from build123d import *

# Parameters (mm, degrees)
SKETCH_1_W          = 150
SKETCH_1_H          = 110
EXTRUDE_1_DEPTH     = 2.5
SKETCH_2_R          = 33.915864145
CUT_EXTRUDE_1_DEPTH = 10


with BuildPart() as part:
    # 草图1 → 凸台-拉伸1 (new, symmetric)
    with BuildSketch(Plane.XY):
        Rectangle(SKETCH_1_W, SKETCH_1_H)
    extrude(amount=EXTRUDE_1_DEPTH, both=True)

    # 草图2 → 切除-拉伸1 (cut)
    with BuildSketch(Plane(origin=(0, 0, -2.5), x_dir=(-1, 0, 0), z_dir=(0, 0, -1))):
        Circle(SKETCH_2_R)
    extrude(amount=-CUT_EXTRUDE_1_DEPTH, mode=Mode.SUBTRACT)


solid = part.part
The listing builds one solid part. Answer for the finished solid, in the listing's coordinates (mm). Give positions to 0.01 mm unless a question says otherwise; leave off trailing zeros. Order: outer loops, then holes, each group sorted by start corner. A loop starts at its lowest first (then second) coordinate and runs counter-clockwise, first axis right, second up. Notation, with made-up numbers: (82.5, -31.75) - (133.5, -31.75) arc R24 cw to (133.5, -4.75) - close; hole circle Ø1 at (79, 2.5). An arc over 180 degrees is marked (long way). One line per item, written item: value. Start each with the question number.
1) A cutting plane is placed at B-B on x = 0. Give the vertices of the cut face in (y, z), then the cut area to 3 significant figures.
2) A cutting plane is placed at C-C on z = 1.4. Give the vertices of the cut face in (x, y), then the cut area to 3 significant figures.
3) The mould has two halves that part along X. Classify faces 1 (the face through (75, -1, 0)), 2 (the face through (-34.4, 0.8, 2.5)), 3 (the face through (26.91, -20.64, -0.04)): released by +X, released by -X, zero draft, split by the parting line, or undercut.
4) Find the intervals of material crossed by L1, parallel to Y at x = 0, z = -0.3; L2, parallel to X at y = 13.5, z = -0.95; L3, parallel to Y at x = -4, z = 2.15, in increasing order.
5) A cutting plane is placed at A-A on y = 0. Give the vertices of the cut face in (x, z), then the cut area to 3 significant figures.
Answer sheet:
1. outline: (-55, -2.5) - (-33.92, -2.5) - (-33.92, 2.5) - (-55, 2.5) - close; (33.92, -2.5) - (55, -2.5) - (55, 2.5) - (33.92, 2.5) - close
1. area: 211 mm2
2. outline: (-75, -55) - (75, -55) - (75, 55) - (-75, 55) - close; hole circle Ø67.83 at (0, 0)
2. area: 12,900 mm2
3. face 1: released by +X
3. face 2: zero draft
3. face 3: undercut
4. L1: y = -55 to -33.92, 33.92 to 55
4. L2: x = -75 to -31.11, 31.11 to 75
4. L3: y = -55 to -33.68, 33.68 to 55
5. outline: (-75, -2.5) - (-33.92, -2.5) - (-33.92, 2.5) - (-75, 2.5) - close; (33.92, -2.5) - (75, -2.5) - (75, 2.5) - (33.92, 2.5) - close
5. area: 411 mm2
